The listing builds one solid part. Answer for the finished solid, in the listing's coordinates (mm). Face numbers are marked on the shaded views. Give positions to 0.01 mm unless a question says otherwise; leave off trailing zeros. Write each loop counter-clockwise with the first axis right and the second up, starting at its lowest first coordinate (ties: lowest second). Pieces come first, ordered by that corner, then holes. Notation, with made-up numbers: (-14, -35) - (22, -35) arc R24 ccw to (22, -14) - close; hole circle Ø2 at (-28.5, 10.5). An arc over 180 degrees is marked (long way). Return JSON: item names as keys, results as strings.
from build123d import *

# Parameters (mm, degrees)
SKETCH1_W             = 120
SKETCH1_H             = 120
BOSS_EXTRUDE1_DEPTH   = 10
FILLET1_R             = 7.5
M5_TAPPED_HOLE1_D     = 4.2
M5_TAPPED_HOLE1_DEPTH = 12.4
M5_TAPPED_HOLE1_TIP   = 1.2618073
SKETCH4_R             = 50
CUT_EXTRUDE1_DEPTH    = 10
M8_TAPPED_HOLE1_D     = 6.8
M8_TAPPED_HOLE1_DEPTH = 19.75
M8_TAPPED_HOLE1_TIP   = 2.042926105


with BuildPart() as part:
    # Sketch1 → Boss-Extrude1 (new body)
    with BuildSketch(Plane.XY):
        Rectangle(SKETCH1_W, SKETCH1_H)
    extrude(amount=BOSS_EXTRUDE1_DEPTH)

    # Fillet1
    fillet1_edges = [part.edges().sort_by_distance(p)[0] for p in [
        (-60, 60, 5),
        (60, 60, 5),
        (60, -60, 5),
        (-60, -60, 5),
    ]]
    fillet(fillet1_edges, radius=FILLET1_R)

    # M5 Tapped Hole1
    with Locations(Plane(origin=(0, 60, 0), x_dir=(1, 0, 0), z_dir=(0, 1, 0))):
        with Locations((-25, -5), (25, -5)):
            Hole(M5_TAPPED_HOLE1_D / 2, depth=M5_TAPPED_HOLE1_DEPTH)
            with Locations((0, 0, -(M5_TAPPED_HOLE1_DEPTH + M5_TAPPED_HOLE1_TIP / 2))):  # 118° drill point
                Cone(0, M5_TAPPED_HOLE1_D / 2, M5_TAPPED_HOLE1_TIP, mode=Mode.SUBTRACT)

    # Sketch4 → Cut-Extrude1 (cut)
    with BuildSketch(Plane.XY.offset(10)):
        Circle(SKETCH4_R)
    extrude(amount=-CUT_EXTRUDE1_DEPTH, mode=Mode.SUBTRACT)

    # M8 Tapped Hole1
    with Locations(Plane.XY.offset(10)):
        with Locations((-45.961940777, 45.961940777), (45.961940777, 45.961940777), (45.961940777, -45.961940777), (-45.961940777, -45.961940777)):
            Hole(M8_TAPPED_HOLE1_D / 2, depth=M8_TAPPED_HOLE1_DEPTH)
            with Locations((0, 0, -(M8_TAPPED_HOLE1_DEPTH + M8_TAPPED_HOLE1_TIP / 2))):  # 118° drill point
                Cone(0, M8_TAPPED_HOLE1_D / 2, M8_TAPPED_HOLE1_TIP, mode=Mode.SUBTRACT)


solid = part.part
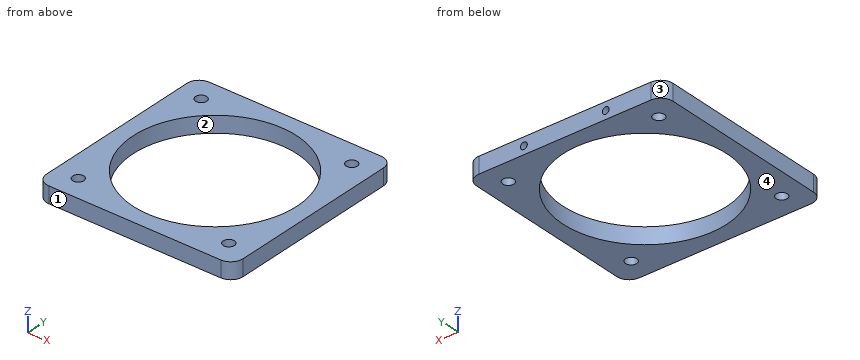
Item 1: A flat-ended cylindrical pin translates along its axis: P1, Ø4, axis at x = -45.96, y = 45.96, coming from the -Z side. Find the tip coordinate at first contact, or state that the pin passes through.
Answer below:
{"P1": "passes through"}
Item 2: A cutting plane is placed at A-A on y = 0. Determine the outline of the cut face in (x, z), then the cut area to 3 significant figures.
Answer below:
{"outline": "(-60, 0) - (-50, 0) - (-50, 10) - (-60, 10) - close; (50, 0) - (60, 0) - (60, 10) - (50, 10) - close", "area": "200 mm²"}
Item 3: A cutting plane is placed at C-C on x = 47. Determine the outline of the cut face in (y, z), then the cut area to 3 significant figures.
Answer below:
{"outline": "(-60, 0) - (-49.2, 0) - (-49.2, 10) - (-60, 10) - close; (-42.72, 0) - (-17.06, 0) - (-17.06, 10) - (-42.72, 10) - close; (17.06, 0) - (42.72, 0) - (42.72, 10) - (17.06, 10) - close; (49.2, 0) - (60, 0) - (60, 10) - (49.2, 10) - close", "area": "729 mm²"}
Item 4: The mould has two halves that part along Y. Classify the marked faces 1, 2, 3 and 4: +Y half, -Y half, draft (parallel to the pull), parting line (faces both ways), or undercut.
Answer below:
{"face 1": "-Y half", "face 2": "undercut", "face 3": "+Y half", "face 4": "draft"}
Item 5: Consider L1, parallel to Y at x = 0, z = 4; L2, parallel to Z at x = -25, y = 55; L3, parallel to X at y = 55, z = 6. Determine where each line is inside the solid, lowest interval first.
Answer below:
{"L1": "y = -60 to -50, 50 to 60", "L2": "z = 0 to 2.9, 7.1 to 10", "L3": "x = -59.57 to -26.85, -23.15 to 23.15, 26.85 to 59.57"}
